```python
from build123d import *

# Parameters (mm, degrees)
FLANGE_PROFILE_SKETCH_R   = 3.5
FLANGE_BODY_25MM_DEPTH    = 25
THROUGH_HOLES_SKETCH_R    = 7
THROUGH_HOLES_DEPTH       = 25
ANNULAR_POCKET_15MM_DEPTH = 15
CROSS_HUB_15MM_DEPTH      = 15


with BuildPart() as part:
    # Flange Profile Sketch → Flange Body 25mm (new body)
    with BuildSketch(Plane.XY):
        with BuildLine():
            ThreePointArc((-7.984837703, 64.507692308), (-32.5, 56.291651246), (-51.872881427, 39.168918449))
            ThreePointArc((-51.872881427, 39.168918449), (-63.219854476, 36.5), (-59.857719129, 25.338773858))
            ThreePointArc((-59.857719129, 25.338773858), (-65, 0), (-59.857719129, -25.338773858))
            ThreePointArc((-59.857719129, -25.338773858), (-63.219854476, -36.5), (-51.872881427, -39.168918449))
            ThreePointArc((-51.872881427, -39.168918449), (-32.5, -56.291651246), (-7.984837703, -64.507692308))
            ThreePointArc((-7.984837703, -64.507692308), (0, -73), (7.984837703, -64.507692308))
            ThreePointArc((7.984837703, -64.507692308), (32.5, -56.291651246), (51.872881427, -39.168918449))
            ThreePointArc((51.872881427, -39.168918449), (63.219854476, -36.5), (59.857719129, -25.338773858))
            ThreePointArc((59.857719129, -25.338773858), (65, 0), (59.857719129, 25.338773858))
            ThreePointArc((59.857719129, 25.338773858), (63.219854476, 36.5), (51.872881427, 39.168918449))
            ThreePointArc((51.872881427, 39.168918449), (32.5, 56.291651246), (7.984837703, 64.507692308))
            ThreePointArc((7.984837703, 64.507692308), (0, 73), (-7.984837703, 64.507692308))
        make_face()
        with Locations((0, 65)):
            Circle(FLANGE_PROFILE_SKETCH_R, mode=Mode.SUBTRACT)
        with Locations((56.291651246, 32.5)):
            Circle(FLANGE_PROFILE_SKETCH_R, mode=Mode.SUBTRACT)
        with Locations((56.291651246, -32.5)):
            Circle(FLANGE_PROFILE_SKETCH_R, mode=Mode.SUBTRACT)
        with Locations((0, -65)):
            Circle(FLANGE_PROFILE_SKETCH_R, mode=Mode.SUBTRACT)
        with Locations((-56.291651246, -32.5)):
            Circle(FLANGE_PROFILE_SKETCH_R, mode=Mode.SUBTRACT)
        with Locations((-56.291651246, 32.5)):
            Circle(FLANGE_PROFILE_SKETCH_R, mode=Mode.SUBTRACT)
    extrude(amount=FLANGE_BODY_25MM_DEPTH)

    # Through Holes Sketch → Through Holes (cut)
    with BuildSketch(Plane.XY.offset(25)):
        with Locations((46, 0)):
            Circle(THROUGH_HOLES_SKETCH_R)
        with Locations(Location((-46, 0, 0), (0, 0, 180))):
            Circle(THROUGH_HOLES_SKETCH_R)
    extrude(amount=-THROUGH_HOLES_DEPTH, mode=Mode.SUBTRACT)

    # Annular Pocket Sketch → Annular Pocket 15mm (cut)
    with BuildSketch(Plane.XY.offset(25)):
        with BuildLine():
            ThreePointArc((43.217391304, 15.756176213), (0, 46), (-43.217391304, 15.756176213))
            ThreePointArc((-43.217391304, 15.756176213), (-30, 0), (-43.217391304, -15.756176213))
            ThreePointArc((-43.217391304, -15.756176213), (0, -46), (43.217391304, -15.756176213))
            ThreePointArc((43.217391304, -15.756176213), (30, 0), (43.217391304, 15.756176213))
        make_face()
    extrude(amount=-ANNULAR_POCKET_15MM_DEPTH, mode=Mode.SUBTRACT)

    # Cross Hub Sketch → Cross Hub 15mm (add)
    with BuildSketch(Plane.XY.offset(10)):
        with BuildLine():
            Line((-7.304627147, 18.618335646), (-16.252048051, 27.56575655))
            ThreePointArc((-16.252048051, 27.56575655), (-22.627416998, 22.627416998), (-27.56575655, 16.252048051))
            Line((-27.56575655, 16.252048051), (-18.618335646, 7.304627147))
            ThreePointArc((-18.618335646, 7.304627147), (-20, 0), (-18.618335646, -7.304627147))
            Line((-18.618335646, -7.304627147), (-27.56575655, -16.252048051))
            ThreePointArc((-27.56575655, -16.252048051), (-22.627416998, -22.627416998), (-16.252048051, -27.56575655))
            Line((-16.252048051, -27.56575655), (-7.304627147, -18.618335646))
            ThreePointArc((-7.304627147, -18.618335646), (0, -20), (7.304627147, -18.618335646))
            Line((7.304627147, -18.618335646), (16.252048051, -27.56575655))
            ThreePointArc((16.252048051, -27.56575655), (22.627416998, -22.627416998), (27.56575655, -16.252048051))
            Line((27.56575655, -16.252048051), (18.618335646, -7.304627147))
            ThreePointArc((18.618335646, -7.304627147), (20, 0), (18.618335646, 7.304627147))
            Line((18.618335646, 7.304627147), (27.56575655, 16.252048051))
            ThreePointArc((27.56575655, 16.252048051), (22.627416998, 22.627416998), (16.252048051, 27.56575655))
            Line((16.252048051, 27.56575655), (7.304627147, 18.618335646))
            ThreePointArc((7.304627147, 18.618335646), (0, 20), (-7.304627147, 18.618335646))
        make_face()
    extrude(amount=CROSS_HUB_15MM_DEPTH)


solid = part.part
```
Verification items for the finished model (mm, model axes). A direction names the side the tool comes from. Give positions to 0.01 mm unless a question says otherwise; leave off trailing zeros. Order: outer loops, then holes, each group sorted by start corner. A loop starts at its lowest first (then second) coordinate and runs counter-clockwise, first axis right, second up. Notation, with made-up numbers: M -39,19.5 L -16,19.5 A23 ccw -16,36.5 Z; hole C 69.25,81 d5. An arc over 180 degrees is marked long. Return JSON: item names as keys, results as strings. Group by question number.
1) Mould release check, pull along Y, two halves, no side actions. Record for faces 1 (the face through (11.841, 23.155, 17.395)), 2 (the face through (-0.786, -45.993, 17.605)), 3 (the face through (0, 0, 25)): pulls with the +Y half, pulls with the -Y half, needs draft (parallel to the pull), parting line crosses it, or undercut.
2) Go/stop test with flat-tipped pins: pin 1 Ø1 at (y, z) = (-52.5, 3.5) entering from -X; pin 2 Ø3 at (y, z) = (-54.5, 22) entering from -X; pin 3 Ø12 at (x, z) = (-42, 18) entering from +Y; pin 4 Ø8.5 at (x, y) = (46, 0) entering from -Z. Record where each tip stops, or that it passes through.
3) Section check A-A on z = 7. Give the number of separate pieces and of enclosed holes in the cut face, and give its area (3 significant figures).
4) Scan lines: line 1 (Y direction, x = -9.5, z = 16); line 2 (Y direction, x = 59.5, z = 13.25); line 3 (X direction, y = 18.5, z = 15). Record each from-to range of solid material in increasing order.
5) Section check C-C on x = 0. Record the cut outline in (y, z), and give its area (3 significant figures).
6) Access from +Z, -Z, +X, -X, +Y, -Y to the whole of each face (thin tool, end or side, straight path). Record for faces 4 (the face through (65, 0, 12)), 5 (the face through (22.547, -22.707, 17.395)).
7) Section check B-B on y = -32.5. Record the cut outline in (x, z), and give its area (3 significant figures).
Answer block:
{
 "1": {"face 1": "undercut", "face 2": "undercut", "face 3": "needs draft"},
 "2": {"pin 1": "stops at x = -39", "pin 2": "stops at x = -37.63", "pin 3": "stops at y = 54.12", "pin 4": "passes through"},
 "3": {"separate pieces": "1", "enclosed holes": "8", "area": "13,400 mm^2"},
 "4": {"line 1": "y = -64.3 to -45.01, -20.81 to 20.81, 45.01 to 64.3", "line 2": "y = -39.83 to -33.9, -31.1 to 31.1, 33.9 to 39.83", "line 3": "x = -62.31 to -42.12, -26.11 to 26.11, 42.12 to 62.31"},
 "5": {"outline": "M -73,0 L -68.5,0 L -68.5,25 L -73,25 Z; M -61.5,0 L 61.5,0 L 61.5,25 L 46,25 L 46,10 L 20,10 L 20,25 L -20,25 L -20,10 L -46,10 L -46,25 L -61.5,25 Z; M 68.5,0 L 73,0 L 73,25 L 68.5,25 Z", "area": "2,520 mm^2"},
 "6": {"face 4": "+Z, -Z, +X", "face 5": "+Z"},
 "7": {"outline": "M -64.29,0 L -59.79,0 L -59.79,25 L -64.29,25 Z; M -52.79,0 L 52.79,0 L 52.79,25 L 32.55,25 L 32.55,10 L -32.55,10 L -32.55,25 L -52.79,25 Z; M 59.79,0 L 64.29,0 L 64.29,25 L 59.79,25 Z", "area": "1,890 mm^2"}
}
